Build history of the part. All positions in model axes, mm. A direction names the side the tool comes from. Give positions to 0.01 mm unless a question says otherwise; leave off trailing zeros. Order: outer loops, then holes, each group sorted by start corner. A loop starts at its lowest first (then second) coordinate and runs counter-clockwise, first axis right, second up. Notation, with made-up numbers: (68, 78) - (117, 78) arc R16 cw to (117, 86) - close; hole circle Ø3 at (37.25, -10). An arc over 180 degrees is marked (long way). Use a Markdown table: item, result. Add a question column.
(1) Mould opens along Z. For faces 1 (the face through (35, -71, 0)), 2 (the face through (48.1, -110, 5.7)), 3 (the face through (55.042, -4.918, 19.113)), 4 (the face through (29, -14, -14)) say: +Z half, -Z half, draft (parallel to the pull), parting line (faces both ways), or undercut.
(2) Flat gauge pins, fed straight in: pin 1 (12 mm diameter, centred on x = 27, y = -22, fed in from +Z); pin 2 (5 mm diameter, centred on x = 23, z = -20.5, fed in from +Y); pin 3 (12 mm diameter, centred on y = -71.5, z = -1, fed in from -X); pin 4 (7 mm diameter, centred on y = -55, z = 28, fed in from -X). Where does each tip first touch, or does it go through?
(3) Which spindle directions (+Z, -Z, +X, -X, +Y, -Y) get a long thin tool onto all of the face, cutting with end or side? Do faces 5 (the face through (26, -46, 3)), 6 (the face through (55.04, -16.25, 38.34)), 7 (the face through (52, -66, 19)), 8 (the face through (29, 5, -28)). Say none if no direction does.
(4) Slice it at B-B (y = -12). Write the cut outline in (x, z), then the cut area to 3 significant figures.
(5) Slice it at D-D (y = -95). Write the cut outline in (x, z), then the cut area to 3 significant figures.
(6) Slice it at A-A (z = 4). Write the cut outline in (x, y).
(7) Slice it at C-C (x = 24). Write the cut outline in (y, z).
(8) Wall check: line 1 (X direction, y = -75.5, z = 30); line 2 (Z direction, x = 37.5, y = -75); line 3 (Z direction, x = 38, y = -9). Give the ranges that are in metal, low to high.
from build123d import *

# Parameters (mm, degrees)
WALL_PLATE_DEPTH           = 6
SIDE_WEB_SKETCH_R          = 6
SIDE_WEB_DEPTH             = 6
CLAMP_BLOCK_SKETCH_W       = 52
CLAMP_BLOCK_SKETCH_H       = 10
CLAMP_BLOCK_DEPTH          = 16
CLAMP_BLOCK_CUT_DEPTH      = 93.11405973
CLAMP_BLOCK_CUT_DEPTH_BACK = 16
U_SADDLE_DEPTH             = 58
LIGHTENING_WINDOW_DEPTH    = 20
HOLE_SKETCH_R              = 10
HOLE_CUT_DEPTH             = 10


with BuildPart() as part:
    # Wall Plate Sketch → Wall Plate (new body)
    with BuildSketch(Plane.XY):
        with BuildLine():
            Line((0, 0), (0, -60))
            Line((0, -60), (13.238780172, -96.774389365))
            ThreePointArc((13.238780172, -96.774389365), (20.556262919, -106.362881582), (32.056528409, -110))
            Line((32.056528409, -110), (38, -110))
            Line((38, -110), (58, -110))
            Line((58, -110), (58, 0))
            Line((58, 0), (0, 0))
        make_face()
    extrude(amount=WALL_PLATE_DEPTH)

    # Side Web Sketch → Side Web (add)
    with BuildSketch(Plane(origin=(58, 0, 0), x_dir=(0, 0, -1), z_dir=(1, 0, 0))):
        with BuildLine():
            ThreePointArc((-21, -110), (-28.878172083, -107.051762515), (-32.885223791, -99.655734106))
            Line((-32.885223791, -99.655734106), (-38.894788475, -56.517756263))
            ThreePointArc((-38.894788475, -56.517756263), (-38.82790492, -53.0618372), (-37.691846294, -49.797297297))
            ThreePointArc((-37.691846294, -49.797297297), (-34.599846625, -37.5), (-37.691846294, -25.202702703))
            ThreePointArc((-37.691846294, -25.202702703), (-38.296228327, -16.128607197), (-31.863054321, -9.700640247))
            Line((-31.863054321, -9.700640247), (-6, 0))
            Line((-6, 0), (-6, -110))
            Line((-6, -110), (-21, -110))
        make_face()
        with Locations((-22, -95)):
            Circle(SIDE_WEB_SKETCH_R, mode=Mode.SUBTRACT)
        with Locations((-28, -55)):
            Circle(SIDE_WEB_SKETCH_R, mode=Mode.SUBTRACT)
        with Locations((-28, -20)):
            Circle(SIDE_WEB_SKETCH_R, mode=Mode.SUBTRACT)
    extrude(amount=-SIDE_WEB_DEPTH)

    # Clamp Block Sketch → Clamp Block (add)
    with BuildSketch(Plane.XY.offset(6)):
        with Locations((26, -55)):
            Rectangle(CLAMP_BLOCK_SKETCH_W, CLAMP_BLOCK_SKETCH_H)
    extrude(amount=CLAMP_BLOCK_DEPTH)

    # Clamp Block Cut Sketch → Clamp Block Cut (cut, two sides: drawn at the far end of the back side and taken through both)
    with BuildSketch(Plane(origin=(0, -50, 0), x_dir=(1, 0, 0), z_dir=(0, 1, 0)).offset(-CLAMP_BLOCK_CUT_DEPTH_BACK)):
        Polygon((0, -22), (52, -22), (0, -6), align=None)
    extrude(amount=CLAMP_BLOCK_CUT_DEPTH + CLAMP_BLOCK_CUT_DEPTH_BACK, mode=Mode.SUBTRACT)

    # U Saddle Sketch → U Saddle (add)
    with BuildSketch(Plane.ZY):
        with BuildLine():
            Line((0, -33), (0, 0))
            ThreePointArc((0, 0), (-14, -14), (-28, 0))
            Line((-28, 0), (-28, 11))
            Line((-28, 11), (-33, 11))
            Line((-33, 11), (-33, 0))
            ThreePointArc((-33, 0), (-27.435028843, -13.435028843), (-14, -19))
            ThreePointArc((-14, -19), (-4.100505063, -23.100505063), (0, -33))
        make_face()
    extrude(amount=-U_SADDLE_DEPTH)

    # Lightening Window Sketch → Lightening Window (cut)
    with BuildSketch(Plane.XY.offset(6)):
        with BuildLine():
            Line((18, -20), (33, -20))
            ThreePointArc((33, -20), (37.242640687, -21.757359313), (39, -26))
            Line((39, -26), (39, -40))
            ThreePointArc((39, -40), (37.242640687, -44.242640687), (33, -46))
            Line((33, -46), (18, -46))
            ThreePointArc((18, -46), (13.757359313, -44.242640687), (12, -40))
            Line((12, -40), (12, -26))
            ThreePointArc((12, -26), (13.757359313, -21.757359313), (18, -20))
        make_face()
    extrude(amount=-LIGHTENING_WINDOW_DEPTH, mode=Mode.SUBTRACT)

    # Hole Sketch → Hole Cut (cut)
    with BuildSketch(Plane.XY.offset(6)):
        with Locations((32, -90)):
            Circle(HOLE_SKETCH_R)
    extrude(amount=-HOLE_CUT_DEPTH, mode=Mode.SUBTRACT)


solid = part.part
Solution:
| question | item | result |
|---|---|---|
| 1 | face 1 | -Z half |
| 1 | face 2 | draft |
| 1 | face 3 | +Z half |
| 1 | face 4 | undercut |
| 2 | pin 1 | z = 6 |
| 2 | pin 2 | y = -10.72 |
| 2 | pin 3 | x = 2.01 |
| 2 | pin 4 | through |
| 3 | face 5 | +Z, -Z |
| 3 | face 6 | +Z, +X, -X |
| 3 | face 7 | +Z, -X |
| 3 | face 8 | +Z, +X, -X, +Y |
| 4 | outline | (0, -28.73) - (58, -28.73) - (58, -21.21) - (0, -21.21) - close; (0, -6.79) - (58, -6.79) - (58, 35.55) - (52, 35.55) - (52, 6) - (0, 6) - close |
| 4 | area | 1,360 mm2 |
| 5 | outline | (12.6, 0) - (23.34, 0) - (23.34, 6) - (12.6, 6) - close; (40.66, 0) - (58, 0) - (58, 16) - (52, 16) - (52, 6) - (40.66, 6) - close; (52, 28) - (58, 28) - (58, 33.53) - (52, 33.53) - close |
| 5 | area | 262 mm2 |
| 6 | outline | (0, -60) - (13.24, -96.77) arc R20 ccw to (32.06, -110) - (58, -110) - (58, 0) - (0, 0) - close; hole (12, -40) arc R6 ccw to (18, -46) - (33, -46) arc R6 ccw to (39, -40) - (39, -26) arc R6 ccw to (33, -20) - (18, -20) arc R6 ccw to (12, -26) - close; hole circle Ø20 at (32, -90) |
| 7 | outline | (-108.31, 0) - (-96, 0) - (-96, 6) - (-108.31, 6) - close; (-84, 0) - (-46, 0) - (-46, 6) - (-50, 6) - (-50, 13.38) - (-60, 13.38) - (-60, 6) - (-84, 6) - close; (-20, -8.8) arc R14 cw to (-19, -14) arc R19 ccw to (0, -33) - (11, -33) - (11, -28) - (0, -28) arc R14 cw to (0, 0) - (0, 6) - (-20, 6) - close |
| 8 | line 1 | 52 to 58 |
| 8 | line 2 | 0 to 6 |
| 8 | line 3 | -30.73 to -24.72, -3.28 to 6 |
